from build123d import *

# Parameters (mm, degrees)
SKETCH1_R               = 5
BOSS_EXTRUDE1_DEPTH     = 326
CHAMFER1_SIZE           = 1
CUT_EXTRUDE1_DEPTH      = 327.076678099
CUT_EXTRUDE1_DEPTH_BACK = 327.076678099
SKETCH8_W               = 156.812935598
SKETCH8_H               = 4.242810574
SKETCH8_H_2             = 7.575578147


with BuildPart() as part:
    # Sketch1 → Boss-Extrude1 (new body)
    with BuildSketch(Plane(origin=(0, 0, 0), x_dir=(0, 0, -1), z_dir=(1, 0, 0))):
        Circle(SKETCH1_R)
    extrude(amount=BOSS_EXTRUDE1_DEPTH)

    # Chamfer1
    chamfer1_edges = [part.edges().sort_by_distance(p)[0] for p in [
        (0, 0, 5),
        (326, 0, 5),
    ]]
    chamfer(chamfer1_edges, length=CHAMFER1_SIZE)

    # Sketch8 → Cut-Extrude1 (cut, two sides: drawn at the far end of the back side and taken through both)
    with BuildSketch(Plane.XY.offset(-CUT_EXTRUDE1_DEPTH_BACK)):
        with Locations((413.406467799, 6.021405287)):
            Rectangle(SKETCH8_W, SKETCH8_H)
        with Locations((413.406467799, -6.021405287)):
            Rectangle(SKETCH8_W, SKETCH8_H)
        with Locations((-69.406467799, 7.687789074)):
            Rectangle(SKETCH8_W, SKETCH8_H_2)
        with Locations((-69.406467799, -7.687789074)):
            Rectangle(SKETCH8_W, SKETCH8_H_2)
    extrude(amount=CUT_EXTRUDE1_DEPTH + CUT_EXTRUDE1_DEPTH_BACK, mode=Mode.SUBTRACT)


solid = part.part
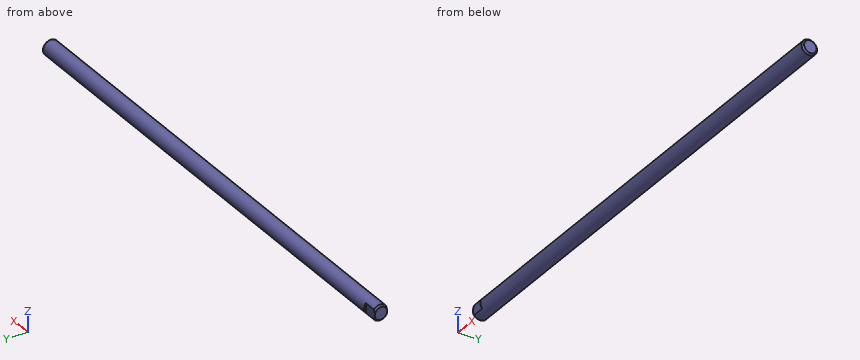
Design review of the part built by this model. Coordinates are the model's own, in mm. Coordinates: 2 decimals unless noted, no trailing zeros. Loops run counter-clockwise (first coordinate to the right, second up) from the corner with the lowest first, then second, coordinate; pieces in that order, holes last. Notation, with made-up numbers: (53, 38.5) - (96, 38.5) arc R10 ccw to (96, 47.5) - close; hole circle Ø10 at (-21, 89.25). An arc over 180 degrees is marked (long way). Use CSV: the item, a comma, the result in double quotes. Start each with the question number.
1. Add section A-A on x = 117.5. Give the boundary of the cut face in (y, z), plus the area to 3 significant figures.
2. To check wall thickness, follow probe 1 along Y at (x, z) = (76, -0.75); probe 2 along Z at (x, y) = (279, 0.5); probe 3 along Y at (x, z) = (75, -3). State the ranges of each line that lie inside material, in increasing order.
3. Clearance check with flat-ended pins moving along their axes: pin 1 (1.9 mm diameter, centred on x = 4.5, z = 0, fed in from +Y); pin 2 (2 mm diameter, centred on x = 172, z = 2.5, fed in from +Y); pin 3 (1.9 mm diameter, centred on x = 3.5, z = 1, fed in from -Y). State where each tip first meets the part, or that it passes through.
Resolved:
1,outline,"circle Ø10 at (0, 0)"
1,area,"78.5 mm2"
2,probe 1,"-4.94 to 4.94"
2,probe 2,"-4.97 to 4.97"
2,probe 3,"-4 to 4"
3,pin 1,"y = 3.9"
3,pin 2,"y = 4.77"
3,pin 3,"y = -3.9"
